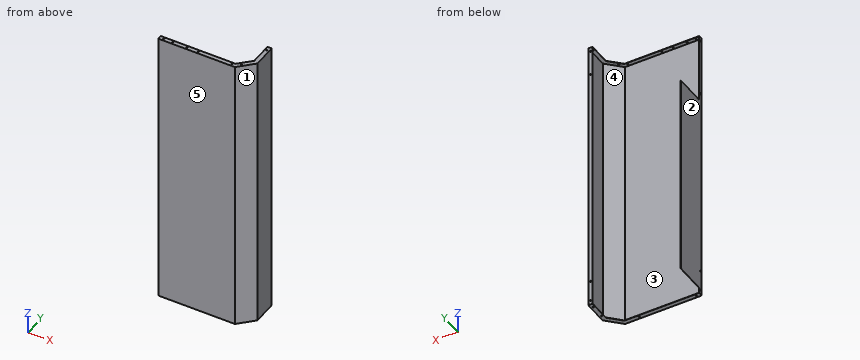
```python
from build123d import *

# Parameters (mm, degrees)
EXTRUDE_1_DEPTH     = 2005
EXTRUDE_1_2_DEPTH   = 28
SKETCH_5_W          = 2
SKETCH_5_H          = 139.764501987
EXTRUDE_2_DEPTH     = 28
SKETCH_6_W          = 540.171572875
SKETCH_6_H          = 2
EXTRUDE_3_DEPTH     = 28
SKETCH_7_W          = 2
SKETCH_7_H          = 2005
EXTRUDE_4_DEPTH     = 28
SKETCH_8_W          = 2
SKETCH_8_H          = 1467
EXTRUDE_5_DEPTH     = 220
SKETCH_9_R          = 4.5
CUT_EXTRUDE_1_DEPTH = 10
SKETCH_11_R         = 4.5
CUT_EXTRUDE_2_DEPTH = 10
SKETCH_12_R         = 4.5
CUT_EXTRUDE_3_DEPTH = 116
SKETCH_13_R         = 4.5
CUT_EXTRUDE_4_DEPTH = 63
SKETCH_14_R         = 4.5
CUT_EXTRUDE_5_DEPTH = 72
CUT_EXTRUDE_START   = -2
SKETCH_15_R         = 4.5
CUT_EXTRUDE_6_DEPTH = 2


with BuildPart() as part:
    # 草图1 → Extrude 1 (new body)
    with BuildSketch(Plane.XY):
        Polygon((0, 0), (541, 0), (641, 100), (641, 270), (639, 270), (639, 100.828427125), (540.171572875, 2), (0, 2), align=None)
    extrude(amount=EXTRUDE_1_DEPTH)

    # 草图4 → Extrude 1 2 (add)
    with BuildSketch(Plane.ZY.offset(-639)):
        Polygon((0, 100.828427125), (0, 270), (2005, 270), (2005, 100.828427125), (2003, 100.828427125), (2003, 268), (2, 268), (2, 100.828427125), align=None)
    extrude(amount=EXTRUDE_1_2_DEPTH)

    # 草图5 → 凸台-拉伸2 (add)
    with BuildSketch(Plane(origin=(269.085786438, -269.085786438, 0), x_dir=(0, 0, 1), z_dir=(-0.7071067811865476, 0.7071067811865476, 0))):
        with Locations((1, 453.255446741)):
            Rectangle(SKETCH_5_W, SKETCH_5_H)
        with Locations((2004, 453.255446741)):
            Rectangle(SKETCH_5_W, SKETCH_5_H)
    extrude(amount=EXTRUDE_2_DEPTH)

    # 草图6 → 凸台-拉伸3 (add)
    with BuildSketch(Plane(origin=(0, 2, 0), x_dir=(1, 0, 0), z_dir=(0, 1, 0))):
        with Locations((270.085786438, -1)):
            Rectangle(SKETCH_6_W, SKETCH_6_H)
        with Locations((270.085786438, -2004)):
            Rectangle(SKETCH_6_W, SKETCH_6_H)
    extrude(amount=EXTRUDE_3_DEPTH)

    # 草图7 → 凸台-拉伸4 (add)
    with BuildSketch(Plane(origin=(0, 2, 0), x_dir=(1, 0, 0), z_dir=(0, 1, 0))):
        with Locations((1, -1002.5)):
            Rectangle(SKETCH_7_W, SKETCH_7_H)
    extrude(amount=EXTRUDE_4_DEPTH)

    # 草图8 → 凸台-拉伸5 (add)
    with BuildSketch(Plane(origin=(0, 30, 0), x_dir=(1, 0, 0), z_dir=(0, 1, 0))):
        with Locations((1, -773.5)):
            Rectangle(SKETCH_8_W, SKETCH_8_H)
    extrude(amount=EXTRUDE_5_DEPTH)

    # 草图9 → 切除-拉伸1 (cut)
    with BuildSketch(Plane.XY.offset(2)):
        with Locations((625, 240)):
            Circle(SKETCH_9_R)
        with Locations((30, 16)):
            Circle(SKETCH_9_R)
        with Locations((431, 16)):
            Circle(SKETCH_9_R)
        with Locations((625, 140)):
            Circle(SKETCH_9_R)
    extrude(amount=-CUT_EXTRUDE_1_DEPTH, mode=Mode.SUBTRACT)

    # 草图11 → 切除-拉伸2 (cut)
    with BuildSketch(Plane.XZ.offset(-268)):
        with Locations(Location((625, 30, 0), (0, 0, 270))):
            Circle(SKETCH_11_R)
        with Locations(Location((625, 180, 0), (0, 0, 270))):
            Circle(SKETCH_11_R)
    extrude(amount=-CUT_EXTRUDE_2_DEPTH, mode=Mode.SUBTRACT)

    # 草图12 → 切除-拉伸3 (cut)
    with BuildSketch(Plane(origin=(2, 0, 0), x_dir=(0, 0, -1), z_dir=(1, 0, 0))):
        with Locations((-30, 16)):
            Circle(SKETCH_12_R)
        with Locations((-180, 16)):
            Circle(SKETCH_12_R)
    extrude(amount=-CUT_EXTRUDE_3_DEPTH, mode=Mode.SUBTRACT)

    # 草图13 → 切除-拉伸4 (cut)
    with BuildSketch(Plane.XZ.offset(-268)):
        with Locations(Location((625, 1975, 0), (0, 0, 270))):
            Circle(SKETCH_13_R)
        with Locations(Location((625, 1795, 0), (0, 0, 270))):
            Circle(SKETCH_13_R)
    extrude(amount=-CUT_EXTRUDE_4_DEPTH, mode=Mode.SUBTRACT)

    # 草图14 → 切除-拉伸5 (cut)
    with BuildSketch(Plane(origin=(2, 0, 0), x_dir=(0, 0, -1), z_dir=(1, 0, 0))):
        with Locations((-1975, 16)):
            Circle(SKETCH_14_R)
        with Locations((-1563, 16)):
            Circle(SKETCH_14_R)
    extrude(amount=-CUT_EXTRUDE_5_DEPTH, mode=Mode.SUBTRACT)

    # 草图15 → 切除-拉伸6 (cut)
    with BuildSketch(Plane(origin=(0, 0, 2003), x_dir=(-1, 0, 0), z_dir=(0, 0, -1)).offset(CUT_EXTRUDE_START)):
        with Locations(Location((-625, 240, 0), (0, 0, 180))):
            Circle(SKETCH_15_R)
        with Locations((-561.360389693, 42.987806691)):
            Circle(SKETCH_15_R)
        with Locations(Location((-30, 16, 0), (0, 0, 180))):
            Circle(SKETCH_15_R)
        with Locations((-511, 16)):
            Circle(SKETCH_15_R)
        with Locations((-273, 16)):
            Circle(SKETCH_15_R)
        with Locations((-193, 16)):
            Circle(SKETCH_15_R)
        with Locations((-93, 16)):
            Circle(SKETCH_15_R)
    extrude(amount=CUT_EXTRUDE_6_DEPTH, mode=Mode.SUBTRACT)


solid = part.part
```
Part model, mm, in its own coordinate system. Face numbers are marked on the shaded views. A direction names the side the tool comes from. Round coordinates to 2 decimals unless told otherwise and drop trailing zeros. Write each loop counter-clockwise with the first axis right and the second up, starting at its lowest first coordinate (ties: lowest second). Pieces come first, ordered by that corner, then holes. Notation, with made-up numbers: M 72.5,41 L 100.5,41 A26 ccw 100.5,74 Z; hole C 42,44.25 d5. An arc over 180 degrees is marked long. Answer as CSV lines item,"result". Start each with the question number.
1) Which spindle directions (+Z, -Z, +X, -X, +Y, -Y) get a long thin tool onto all of the face, cutting with end or side? Do the marked faces 4 and 5. Say none if no direction does.
2) Mould opens along X. For the marked faces 1, 2 and 3 say: +X half, -X half, draft (parallel to the pull), parting line (faces both ways), or undercut.
3) Band-saw the part on D-D (y = 67). List the corners of the cut face in (x, z), then the cut area to 3 significant figures.
4) Band-saw the part on B-B (x = 242.5). List the corners of the cut face in (y, z), then the cut area to 3 significant figures.
5) Drill centre lines: L1, parallel to Z at x = 625, y = 268.5; L2, parallel to Y at x = 0.65, z = 1975; L3, parallel to X at y = 268.75, z = 30. Where is each one in solid material? Low to high.
6) Band-saw the part on A-A (y = 162). List the corners of the cut face in (x, z), then the cut area to 3 significant figures.
7) Band-saw the part on C-C (z = 400.5). List the corners of the cut face in (x, y), then the cut area to 3 significant figures.
8) Drop flat-ended pins along their axis: pin 1 (1.5 mm diameter, centred on x = 499, z = 261.5, fed in from +Y); pin 2 (0.6 mm diameter, centred on x = 1, z = 1110.5, fed in from +Y); pin 3 (5.5 mm diameter, centred on x = 561.36, y = 42.99, fed in from +Z). Give the stop position or say it passes through.
Worked out:
1,face 4,"none"
1,face 5,"+Z, -Z, +X, -X, -Y"
2,face 1,"+X half"
2,face 2,"-X half"
2,face 3,"undercut"
3,outline,"M 0,40 L 2,40 L 2,1507 L 0,1507 Z; M 565.57,0 L 608,0 L 608,2005 L 565.57,2005 L 565.57,2003 L 605.17,2003 L 605.17,2 L 565.57,2 Z"
3,area,"8,760 mm²"
4,outline,"M 0,0 L 30,0 L 30,2 L 2,2 L 2,2003 L 30,2003 L 30,2005 L 0,2005 Z"
4,area,"4,120 mm²"
5,L1,"0 to 25.5, 34.5 to 175.5, 184.5 to 1790.5, 1799.5 to 1970.5, 1979.5 to 2005"
5,L2,"0 to 11.5, 20.5 to 30"
5,L3,"611 to 620.5, 629.5 to 641"
6,outline,"M 0,40 L 2,40 L 2,1507 L 0,1507 Z; M 611,0 L 641,0 L 641,2005 L 611,2005 L 611,2003 L 639,2003 L 639,2 L 611,2 Z"
6,area,"7,060 mm²"
7,outline,"M 0,0 L 541,0 L 641,100 L 641,270 L 611,270 L 611,268 L 639,268 L 639,100.83 L 540.17,2 L 2,2 L 2,250 L 0,250 Z"
7,area,"2,250 mm²"
8,pin 1,"y = 2"
8,pin 2,"y = 250"
8,pin 3,"z = 2"
